For this review, use the dimensioned drawing (mm, ordinates from the lowest corner) and the shaded views. A direction names the side the tool comes from. Coordinates: 2 decimals unless noted, no trailing zeros. Loops run counter-clockwise (first coordinate to the right, second up) from the corner with the lowest first, then second, coordinate; pieces in that order, holes last. Notation, with made-up numbers: (24.5, 76.25) - (47.5, 76.25) arc R33 ccw to (47.5, 109.25) - close; hole circle Ø10 at (-10, -24.75). An arc over 180 degrees is marked (long way). One line per item, written item: value. Start each with the question number.
1. For the marked faces 1, 2 and 3, list the 3-axis set-ups (+Z, -Z, +X, -X, +Y, -Y) from which the entire face can be reached by the end or side of a thin tool; tool diameter is ignored.
2. Mouldability with a two-part tool opening along Z and no side actions: class the marked faces 4, 5 and 6 as +Z half, -Z half, draft (parallel to the pull), parting line (faces both ways), or undercut.
3. We need section D-D, the plane y = 27. Give the boundary of the cut face in (x, z) (1 decimal).
4. Insertion check: P1, Ø13, axis at y = 50.5, z = 4.5, coming from the +X side; P2, Ø10, axis at x = 67.5, y = 7.5, coming from the +Z side; P3, Ø5, axis at x = 119.5, z = 103, coming from the +Y side. Each pin has a flat end and moves straight along its axis. Give the tip position at first contact, or say it passes through.
5. To check wall thickness, follow line 1 (Z direction, x = 83, y = 14); line 2 (Y direction, x = 85, z = 8); line 3 (Z direction, x = 94.5, y = 39) (1 decimal). State the ranges of each line that lie inside material, in increasing order.
6. We need section C-C, the plane x = 143. Give the boundary of the cut face in (y, z).
7. We need section B-B, the plane y = 54. Give the boundary of the cut face in (x, z) (1 decimal), then the cut area to 3 significant figures.
8. We need section A-A, the plane x = 83. Give the boundary of the cut face in (y, z).
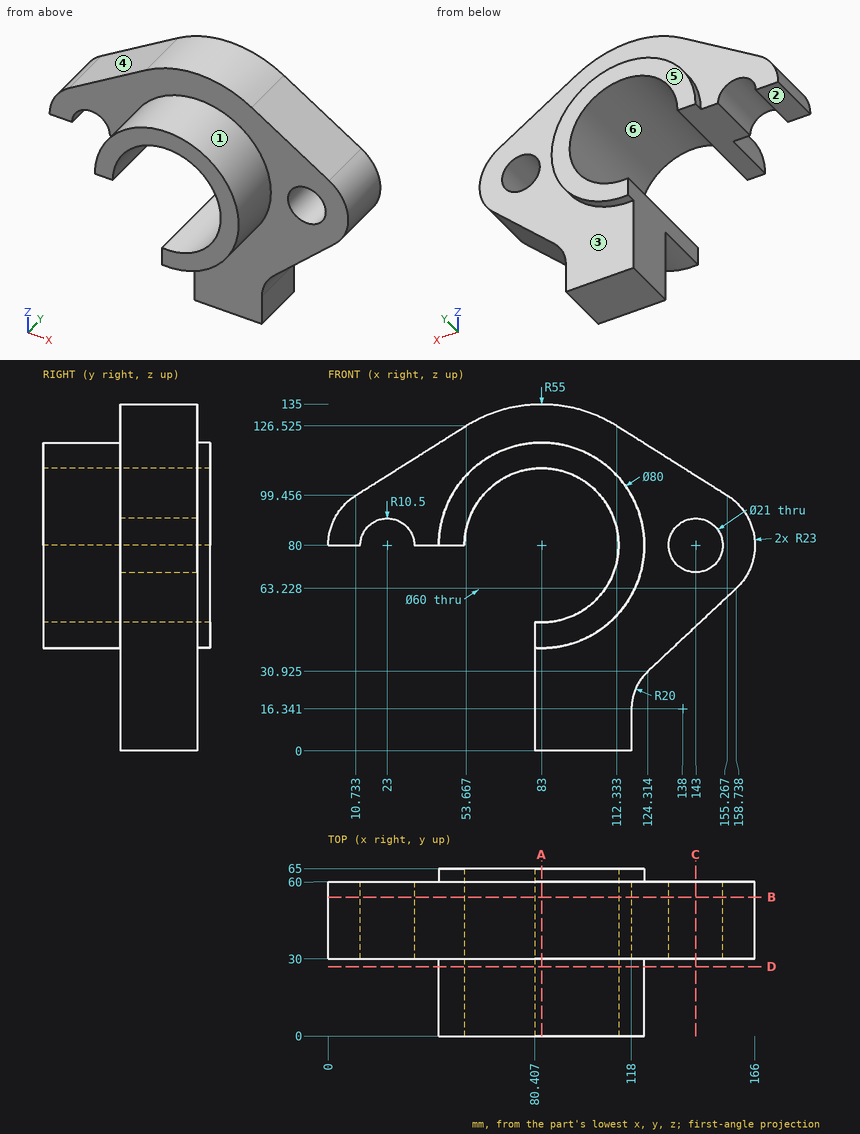
Findings below:
1. face 1: -Y
1. face 2: -Z, -X, +Y, -Y
1. face 3: +Y
2. face 4: +Z half
2. face 5: draft
2. face 6: undercut
3. outline: (43, 80) - (53, 80) arc R30 cw (long way) to (80.4, 50.1) - (80.4, 40.1) arc R40 ccw (long way) to start
4. P1: x = 118
4. P2: z = 118.6
4. P3: y = 60
5. line 1: 40 to 50, 110 to 120
5. line 2: 30 to 60
5. line 3: 0 to 52.3, 107.7 to 133.8
6. outline: (30, 48.46) - (60, 48.46) - (60, 69.5) - (30, 69.5) - close; (30, 90.5) - (60, 90.5) - (60, 107.19) - (30, 107.19) - close
7. outline: (0, 80) - (12.5, 80) arc R10.5 cw to (33.5, 80) - (53, 80) arc R30 cw (long way) to (80.4, 50.1) - (80.4, 0) - (118, 0) - (118, 16.3) arc R20 cw to (124.3, 30.9) - (158.7, 63.2) arc R23 ccw to (155.3, 99.5) - (112.3, 126.5) arc R55 ccw to (53.7, 126.5) - (10.7, 99.5) arc R23 ccw to start; hole circle Ø21 at (143, 80)
7. area: 8,040 mm2
8. outline: (0, 40) - (30, 40) - (30, 0) - (60, 0) - (60, 40) - (65, 40) - (65, 50) - (0, 50) - close; (0, 110) - (65, 110) - (65, 120) - (60, 120) - (60, 135) - (30, 135) - (30, 120) - (0, 120) - close
